Verification items for the finished model (mm, model axes). A direction names the side the tool comes from. Coordinates: 2 decimals unless noted, no trailing zeros. Write each loop counter-clockwise with the first axis right and the second up, starting at its lowest first coordinate (ties: lowest second). Pieces come first, ordered by that corner, then holes.
```python
from build123d import *

# Parameters (mm, degrees)
BLOCK_BODY_EXTRUDE_30MM_DEPTH = 30
POCKET_SKETCH_W               = 20
POCKET_SKETCH_H               = 10
POCKET_CUT_10MM_DEPTH         = 10


with BuildPart() as part:
    # Block Profile Sketch → Block Body Extrude 30mm (new body)
    with BuildSketch(Plane.XY):
        Polygon((0, 0), (0, 40), (15, 40), (15, 55), (35, 55), (35, 40), (50, 40), (50, 0), (30, 0), (30, 10), (40, 10), (40, 30), (10, 30), (10, 10), (20, 10), (20, 0), align=None)
    extrude(amount=BLOCK_BODY_EXTRUDE_30MM_DEPTH)

    # Pocket Sketch → Pocket Cut 10mm (cut)
    with BuildSketch(Plane(origin=(0, 55, 0), x_dir=(1, 0, 0), z_dir=(0, 1, 0))):
        with Locations((25, -15)):
            Rectangle(POCKET_SKETCH_W, POCKET_SKETCH_H)
    extrude(amount=-POCKET_CUT_10MM_DEPTH, mode=Mode.SUBTRACT)


solid = part.part
```
1. Draft check along X on faces 1 (the flat face through (30, 5, 15)), 2 (the flat face through (7, 40, 15)), 3 (the flat face through (50, 20, 15)). Enter one of: pulls with the +X half, pulls with the -X half, needs draft (parallel to the pull), parting line crosses it, or undercut.
2. Sectioned sample at B-B, the plane y = 25. Record the boundary of the cut face in (x, z).
3. Sectioned sample at D-D, the plane x = 22. Record the boundary of the cut face in (y, z).
4. Sectioned sample at C-C, the plane z = 16.75. Record the boundary of the cut face in (x, y).
5. Material ranges on L1, parallel to X at y = 22, z = 24.25; L2, parallel to X at y = 3.5, z = 4.25; L3, parallel to Y at x = 17, z = 3, recorded low to high.
6. Gauge pin test, flat ends, axial feed: P1, Ø1.5, axis at y = 47, z = 23, coming from the -X side; P2, Ø16.5, axis at y = 50, z = 9, coming from the +X side; P3, Ø16, axis at y = 25, z = 17, coming from the -X side; P4, Ø12, axis at x = 44, z = 15, coming from the +Y side. Record the tip position at first contact, or that the pin passes through.
7. Sectioned sample at A-A, the plane x = 37. Record the boundary of the cut face in (y, z), and give its area (3 significant figures).
8. Tool access check on faces 4 (the flat face through (35, 44, 15)), 5 (the flat face through (25, 50, 10)), 6 (the flat face through (15, 44, 15)), 7 (the flat face through (20, 5, 15)), 8 (the flat face through (15, 10, 15)). Record the directions out of +Z, -Z, +X, -X, +Y, -Y that give a thin tool (end or side, any length) a straight path to the whole face; none if there is none.
Outcome:
1. face 1: undercut
1. face 2: needs draft
1. face 3: pulls with the +X half
2. outline: (0, 0) - (10, 0) - (10, 30) - (0, 30) - close; (40, 0) - (50, 0) - (50, 30) - (40, 30) - close
3. outline: (30, 0) - (55, 0) - (55, 10) - (45, 10) - (45, 20) - (55, 20) - (55, 30) - (30, 30) - close
4. outline: (0, 0) - (20, 0) - (20, 10) - (10, 10) - (10, 30) - (40, 30) - (40, 10) - (30, 10) - (30, 0) - (50, 0) - (50, 40) - (35, 40) - (35, 45) - (15, 45) - (15, 40) - (0, 40) - close
5. L1: x = 0 to 10, 40 to 50
5. L2: x = 0 to 20, 30 to 50
5. L3: y = 0 to 10, 30 to 55
6. P1: stops at x = 15
6. P2: stops at x = 35
6. P3: stops at x = 0
6. P4: stops at y = 40
7. outline: (0, 0) - (10, 0) - (10, 30) - (0, 30) - close; (30, 0) - (40, 0) - (40, 30) - (30, 30) - close
7. area: 600 mm2
8. face 4: +Z, -Z, +X, +Y
8. face 5: +X, -X, +Y
8. face 6: +Z, -Z, -X, +Y
8. face 7: +Z, -Z, -Y
8. face 8: +Z, -Z
